```python
from build123d import *


with BuildPart() as part:
    # Shaft Profile Sketch → Stepped Shaft Ø20 Journals Ø12 (revolve)
    with BuildSketch(Plane.XY, mode=Mode.PRIVATE) as stepped_shaft_20_journals_12_sk:
        Polygon((0, 0), (6, 0), (6, 10), (10, 10), (10, 110), (6, 110), (6, 120), (0, 120), align=None)
    revolve(stepped_shaft_20_journals_12_sk.sketch.rotate(Axis((0, 120, 0), (0, -1, 0)), 90), axis=Axis((0, 120, 0), (0, -1, 0)))


solid = part.part
```
Model file for the job. Use its own axes, mm. A direction names the side the tool comes from. Round coordinates to 2 decimals unless told otherwise and drop trailing zeros. Write each loop counter-clockwise with the first axis right and the second up, starting at its lowest first coordinate (ties: lowest second). Pieces come first, ordered by that corner, then holes. Notation, with made-up numbers: (31, 27) - (63, 27) arc R34 cw to (63, 63) - close; hole circle Ø1 at (-15, 22). An arc over 180 degrees is marked (long way). Use CSV: the item, a comma, the result in double quotes. Start each with the question number.
Item 1: Tool access for faces 1 (the face through (0, 0, 0)), 2 (the face through (0, 110, 7)), 3 (the face through (7, 10, 0)): list every direction of +Z, -Z, +X, -X, +Y, -Y with a clear straight run to the whole face (end or side of a thin tool).
Item 2: Drill centre lines: L1, parallel to Y at x = 7.5, z = 5; L2, parallel to Z at x = 0.5, y = 18.5; L3, parallel to Z at x = 8, y = 107.5. Where is each one in solid material? Low to high. Write a range as [from, to].
Item 3: Band-saw the part on C-C (y = 91). Write the cut outline in (x, z), and give its area (3 significant figures).
Item 4: Band-saw the part on D-D (x = 8.75). Write the cut outline in (y, z).
Item 5: Band-saw the part on B-B (z = 0). Write the cut outline in (x, y).
Item 6: Band-saw the part on A-A (x = 0). Write the cut outline in (y, z).
Item 7: Pin check, flat tips, straight feed: P1, Ø5, axis at x = 7.5, y = 95.5, coming from the -Z side; P2, Ø8, axis at x = 6.5, y = 29.5, coming from the +Z side; P3, Ø5, axis at y = 16.5, z = -5.5, coming from the +X side. Stop position of each tip, or through.
Checked values:
1,face 1,"+Z, -Z, +X, -X, -Y"
1,face 2,"+Y"
1,face 3,"-Y"
2,L1,"y = [10, 110]"
2,L2,"z = [-9.99, 9.99]"
2,L3,"z = [-6, 6]"
3,outline,"circle Ø20 at (0, 0)"
3,area,"314 mm²"
4,outline,"(10, -4.84) - (110, -4.84) - (110, 4.84) - (10, 4.84) - close"
5,outline,"(-10, 10) - (-6, 10) - (-6, 0) - (6, 0) - (6, 10) - (10, 10) - (10, 110) - (6, 110) - (6, 120) - (-6, 120) - (-6, 110) - (-10, 110) - close"
6,outline,"(0, -6) - (10, -6) - (10, -10) - (110, -10) - (110, -6) - (120, -6) - (120, 6) - (110, 6) - (110, 10) - (10, 10) - (10, 6) - (0, 6) - close"
7,P1,"stops at z = -8.66"
7,P2,"stops at z = 9.68"
7,P3,"stops at x = 9.54"
